Build history of the part. All positions in model axes, mm. Face numbers are marked on the shaded views. Coordinates: 2 decimals unless noted, no trailing zeros. Loops run counter-clockwise (first coordinate to the right, second up) from the corner with the lowest first, then second, coordinate; pieces in that order, holes last.
Item 1: Mould opens along Z. For the marked faces 1, 2 and 3 say: released by +Z, released by -Z, zero draft, split by the parting line, or undercut.
Item 2: Cut at B-B (x = 0). List the corners of the cut face in (y, z).
Item 3: Flat gauge pins, fed straight in: pin 1 (12 mm diameter, centred on x = -12, y = 1.5, fed in from -Z); pin 2 (1 mm diameter, centred on y = 7, z = -7, fed in from -X); pin 3 (12 mm diameter, centred on y = 0, z = -9.5, fed in from +X). Where does each tip first touch, or does it go through?
Item 4: Drill centre lines: line 1 along X through (y, z) = (-0.25, 0); line 2 along X through (y, z) = (7.5, 1.5); line 3 along Z through (x, y) = (-11, -6.5). Where is each one in solid material? Low to high.
Item 5: Cut at C-C (z = -7.5). List the corners of the cut face in (x, y).
Item 6: Cut at D-D (x = 16.5). List the corners of the cut face in (y, z), and give its area (3 significant figures).
Item 7: Cut at A-A (y = 2.5). List the corners of the cut face in (x, z).
from build123d import *

# Parameters (mm, degrees)
HEX_PROFILE_SKETCH_R = 13
HEX_NUT_BODY_DEPTH   = 10


with BuildPart() as part:
    # Hex Profile Sketch → Hex Nut Body (new, symmetric)
    with BuildSketch(Plane(origin=(0, 0, 0), x_dir=(1, 0, 0), z_dir=(0, 1, 0))):
        Polygon((20.207259422, 0), (10.103629711, 17.5), (-10.103629711, 17.5), (-20.207259422, 0), (-10.103629711, -17.5), (10.103629711, -17.5), align=None)
        with Locations(Location((0, 0, 0), (0, 0, 270))):
            Circle(HEX_PROFILE_SKETCH_R, mode=Mode.SUBTRACT)
    extrude(amount=HEX_NUT_BODY_DEPTH, both=True)

    # Corner Chamfer Profile → Corner Chamfer Cut (revolve, cut)
    with BuildSketch(Plane.XY):
        with BuildLine():
            Line((18.207259422, 10), (20.207259422, 10))
            Line((20.207259422, 10), (20.207259422, 8))
            ThreePointArc((20.207259422, 8), (19.457751072, 9.25049165), (18.207259422, 10))
        make_face()
    revolve(axis=Axis((0, 0, 0), (0, 1, 0)), mode=Mode.SUBTRACT)


solid = part.part
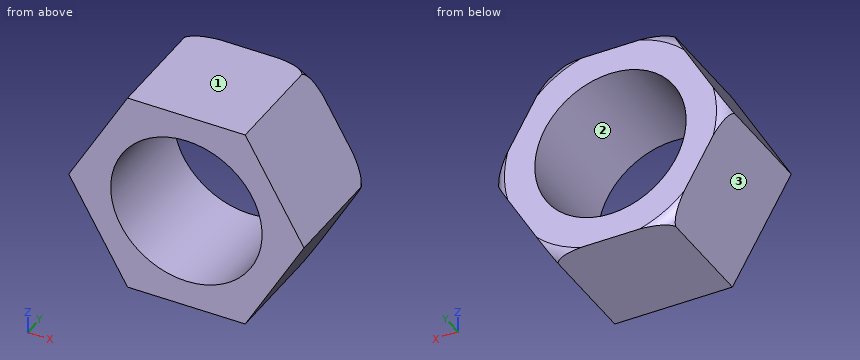
Filled sheet:
1. face 1: released by +Z
1. face 2: undercut
1. face 3: released by -Z
2. outline: (-10, -17.5) - (10, -17.5) - (10, -13) - (-10, -13) - close; (-10, 13) - (10, 13) - (10, 17.5) - (-10, 17.5) - close
3. pin 1: stops at z = -17.5
3. pin 2: stops at x = -16.45
3. pin 3: stops at x = 18.19
4. line 1: x = -20.21 to -13, 13 to 20.21
4. line 2: x = -19.34 to -12.91, 12.91 to 19.34
4. line 3: z = -15.95 to -6.93, 6.93 to 15.95
5. outline: (-15.88, -10) - (-10.62, -10) - (-10.62, 10) - (-15.88, 10) - close; (10.62, -10) - (15.88, -10) - (15.88, 10) - (10.62, 10) - close
6. outline: (-10, -6.42) - (10, -6.42) - (10, 6.42) - (-10, 6.42) - close
6. area: 257 mm2
7. outline: (-20.21, 0) - (-10.1, -17.5) - (10.1, -17.5) - (20.21, 0) - (10.1, 17.5) - (-10.1, 17.5) - close; hole circle Ø26 at (0, 0)
